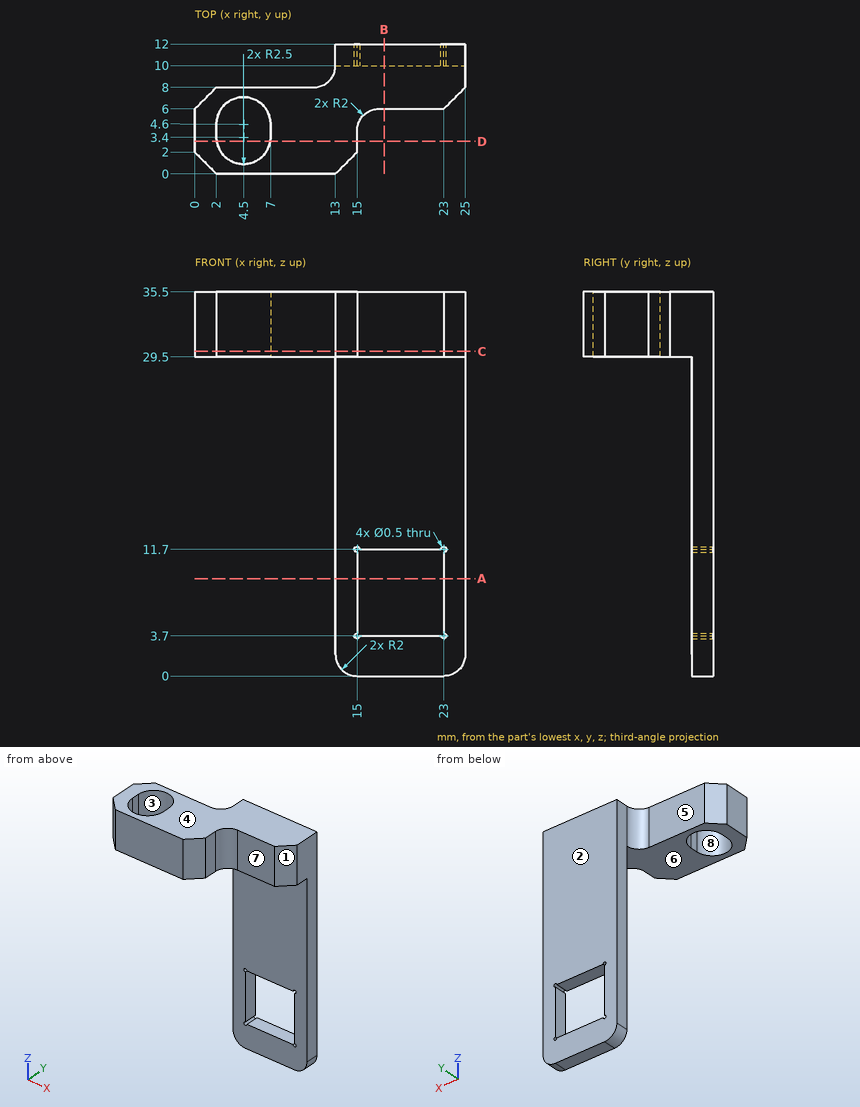
The figure shows three views and two pictorial views of one solid part (mm, origin at its lowest corner). Answer the questions. A direction names the side the tool comes from. Round coordinates to 2 decimals unless told otherwise and drop trailing zeros. Order: outer loops, then holes, each group sorted by start corner. A loop starts at its lowest first (then second) coordinate and runs counter-clockwise, first axis right, second up. Notation, with made-up numbers: (-3.75, -38) - (36.25, -38) arc R19 cw to (36.25, -26) - close; hole circle Ø4 at (4, 88). An arc over 180 degrees is marked (long way). Write item = value, one per line. Start each with the question number.
1) Straight lines are drawn through the part: L1, parallel to Y at x = 14.75, z = 19.5; L2, parallel to X at y = 11.25, z = 12.5; L3, parallel to X at y = 1.5, z = 30.5. For each, find the intervals that lie inside material, in ascending order.
2) Section C-C, the plane z = 30 is taken. Write down the section's boundary in (x, y).
3) Section B-B, the plane x = 17.5 is taken. Write down the section's boundary in (y, z).
4) Section D-D, the plane y = 3 is taken. Write down the section's boundary in (x, z), plus the area to 3 significant figures.
5) Given pin 1 (2 mm diameter, centred on y = 11.5, z = 16, fed in from -X); pin 2 (1 mm diameter, centred on y = 3, z = 32.5, fed in from +X); pin 3 (5 mm diameter, centred on y = 9, z = 16.5, fed in from +X); pin 4 (1.5 mm diameter, centred on x = 19.5, y = 5, fed in from +Z), each flat-ended and moving along its own axis, determine where each tip first touches the part or whether it passes through.
6) For a pull along Y with two mould halves and no side action, classify the marked faces 1, 2 and 3 as released by +Y, released by -Y, zero draft, split by the parting line, or undercut.
7) Section A-A, the plane z = 9 is taken. Write down the section's boundary in (x, y).
8) For the marked faces 4, 5, 6, 7 and 8, determine the directions among +Z, -Z, +X, -X, +Y, -Y from which every point of the face is accessible in a straight line to the end or side of a thin tool.
Results list:
q1.L1 = 10 to 12
q1.L2 = 13 to 25
q1.L3 = 0.5 to 2.88, 6.12 to 14.5
q2.outline = (0, 2) - (2, 0) - (13, 0) - (15, 2) - (15, 4) arc R2 cw to (17, 6) - (23, 6) - (25, 8) - (25, 12) - (13, 12) - (13, 10) arc R2 cw to (11, 8) - (2, 8) - (0, 6) - close; hole (2, 3.4) arc R2.5 ccw to (7, 3.4) - (7, 4.6) arc R2.5 ccw to (2, 4.6) - close
q3.outline = (6, 29.5) - (10, 29.5) - (10, 11.7) - (12, 11.7) - (12, 35.5) - (6, 35.5) - close; (10, 0) - (12, 0) - (12, 3.7) - (10, 3.7) - close
q4.outline = (0, 29.5) - (2.03, 29.5) - (2.03, 35.5) - (0, 35.5) - close; (6.97, 29.5) - (15, 29.5) - (15, 35.5) - (6.97, 35.5) - close
q4.area = 60.4 mm^2
q5.pin_1 = 13
q5.pin_2 = 15
q5.pin_3 = 25
q5.pin_4 = through
q6.face_1 = released by -Y
q6.face_2 = released by +Y
q6.face_3 = undercut
q7.outline = (13, 10) - (15, 10) - (15, 12) - (13, 12) - close; (23, 10) - (25, 10) - (25, 12) - (23, 12) - close
q8.face_4 = +Z, +X, -X, +Y, -Y
q8.face_5 = +Z, -Z, -X, +Y
q8.face_6 = -Z, +X, -X, -Y
q8.face_7 = +Z, -Z, +X, -Y
q8.face_8 = +Z, -Z
